For this review, use the dimensioned drawing (mm, ordinates from the lowest corner) and the shaded views. A direction names the side the tool comes from. Give positions to 0.01 mm unless a question says otherwise; leave off trailing zeros. Order: outer loops, then holes, each group sorted by start corner. A loop starts at its lowest first (then second) coordinate and runs counter-clockwise, first axis right, second up. Notation, with made-up numbers: (-4, 70.25) - (45, 70.25) arc R20 ccw to (45, 96.25) - close; hole circle Ø6 at (1, -16). An arc over 180 degrees is marked (long way). One line per item, written item: value.
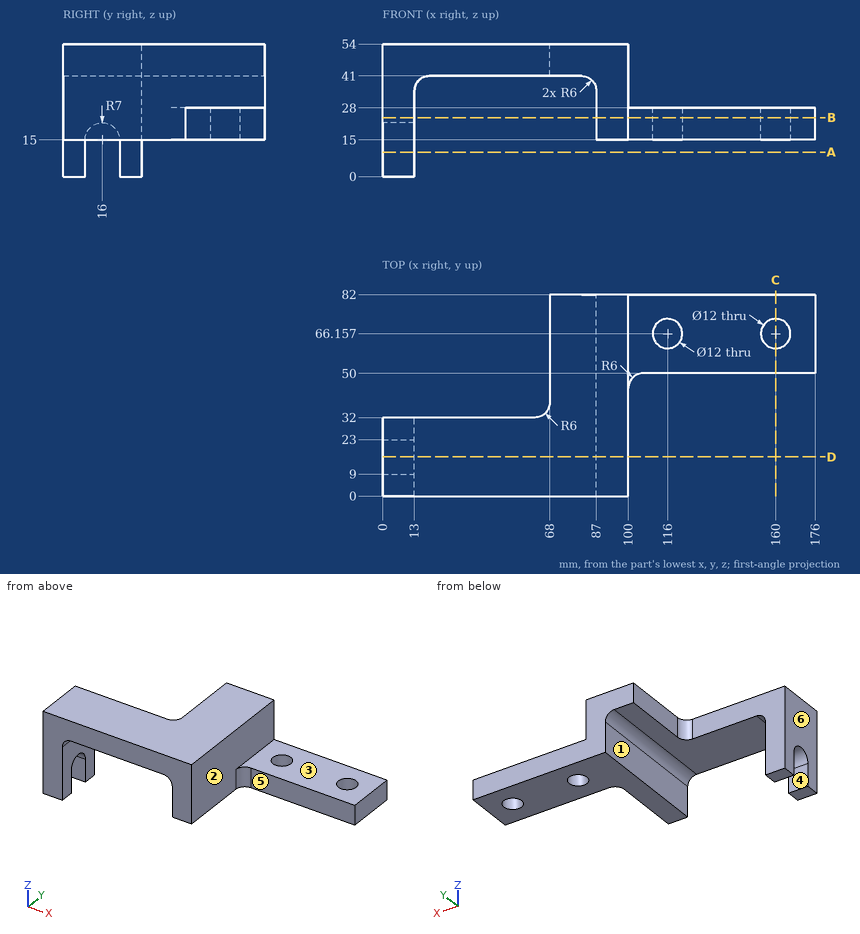
(1) Wall thickness on line 1 (X direction, y = 24, z = 17.5); line 2 (Y direction, x = 160, z = 21.25); line 3 (Y direction, x = 56, z = 46): over which ranges is each line inside the solid? List them lowest first. Write a range as from..to.
Answers below:
line 1: x = 0..13, 87..100
line 2: y = 50..60.16, 72.16..82
line 3: y = 0..32
(2) Take a section at B-B (z = 24). Write out the cut boundary in (x, y), then the cut area to 3 significant figures.
Answers below:
outline: (0, 0) - (13, 0) - (13, 32) - (0, 32) - close; (87, 0) - (100, 0) - (100, 44) arc R6 cw to (106, 50) - (176, 50) - (176, 82) - (87, 82) - close; hole circle Ø12 at (116, 66.16); hole circle Ø12 at (160, 66.16)
area: 3,700 mm^2
(3) For P1, Ø1, axis at y = 63.5, z = 36.5, coming from the +X side; P2, Ø14.5, axis at y = 60, z = 49.5, coming from the -X side; P3, Ø10.5, axis at x = 5, z = 11, coming from the +Y side, all flat-tipped, find the tip position at first contact; note any pin that passes through.
Answers below:
P1: stops at x = 100
P2: stops at x = 68
P3: stops at y = 32
(4) Take a section at C-C (x = 160). Write out the cut boundary in (y, z), then the cut area to 3 significant figures.
Answers below:
outline: (50, 15) - (60.16, 15) - (60.16, 28) - (50, 28) - close; (72.16, 15) - (82, 15) - (82, 28) - (72.16, 28) - close
area: 260 mm^2
(5) Draft analysis for pull direction Y (two halves, no side actions). For the marked faces 4, 5 and 6, state which applies: pulls with the +Y half, pulls with the -Y half, needs draft (parallel to the pull), parting line crosses it, or undercut.
Answers below:
face 4: undercut
face 5: pulls with the -Y half
face 6: needs draft
(6) Take a section at D-D (y = 16). Write out the cut boundary in (x, z), then the cut area to 3 significant figures.
Answers below:
outline: (0, 22) - (13, 22) - (13, 35) arc R6 cw to (19, 41) - (81, 41) arc R6 cw to (87, 35) - (87, 15) - (100, 15) - (100, 54) - (0, 54) - close
area: 1,900 mm^2
(7) Machinability: for the marked faces 1, 2 and 3, which of the approach directions +Z, -Z, +X, -X, +Y, -Y give a long, thin tool a straight path to every point of the face, cutting with its end or side? Answer none if there is none.
Answers below:
face 1: -Z, +Y, -Y
face 2: +Z, +X, -Y
face 3: +Z, +X, +Y, -Y
(8) Take a section at A-A (z = 10). Write out the cut boundary in (x, y).
Answers below:
outline: (0, 0) - (13, 0) - (13, 9) - (0, 9) - close; (0, 23) - (13, 23) - (13, 32) - (0, 32) - close
